Source: three-view drawing plus pictorial views. Frame: mm from the lowest corner of the part. Round coordinates to 2 decimals unless told otherwise and drop trailing zeros. Order: outer loops, then holes, each group sorted by start corner. A loop starts at its lowest first (then second) coordinate and runs counter-clockwise, first axis right, second up. Notation, with made-up numbers: (4, 61.25) - (58, 61.25) arc R15 ccw to (58, 70.25) - close; hole circle Ø9 at (20.5, 18.5). An arc over 180 degrees is marked (long way). Use one line per item in the form item = value. Start each with the question number.
Q1. Draft query along Z for the marked faces 1, 2 and 3. Return one class per face: released by +Z, released by -Z, zero draft, split by the parting line, or undercut.
Q2. Pin query (flat end, axial travel): pin 1 Ø1.5 at (y, z) = (8.5, 9) entering from -X; pin 2 Ø4 at (y, z) = (6, 8) entering from +X; pin 3 Ø1 at (y, z) = (4, 2.5) entering from -X; pin 4 Ø9.5 at (x, z) = (15.01, 13) entering from +Y. Return the tip coordinate at first contact, or that it passes through.
Q3. Cut plane A-A, the plane y = 5.5. Return the cut outline in (x, z) (1 decimal), and give its area (3 significant figures).
Q4. Cut plane B-B, the plane y = 11.5. Return the cut outline in (x, z) (1 decimal).
Q5. Ray query, line 1 (Z direction, x = 14, y = 3.5) (1 decimal); line 2 (Z direction, x = 11, y = 2.5); line 3 (X direction, y = 2.5, z = 13). Return the intervals inside material, ascending. Write a range as [from, to].
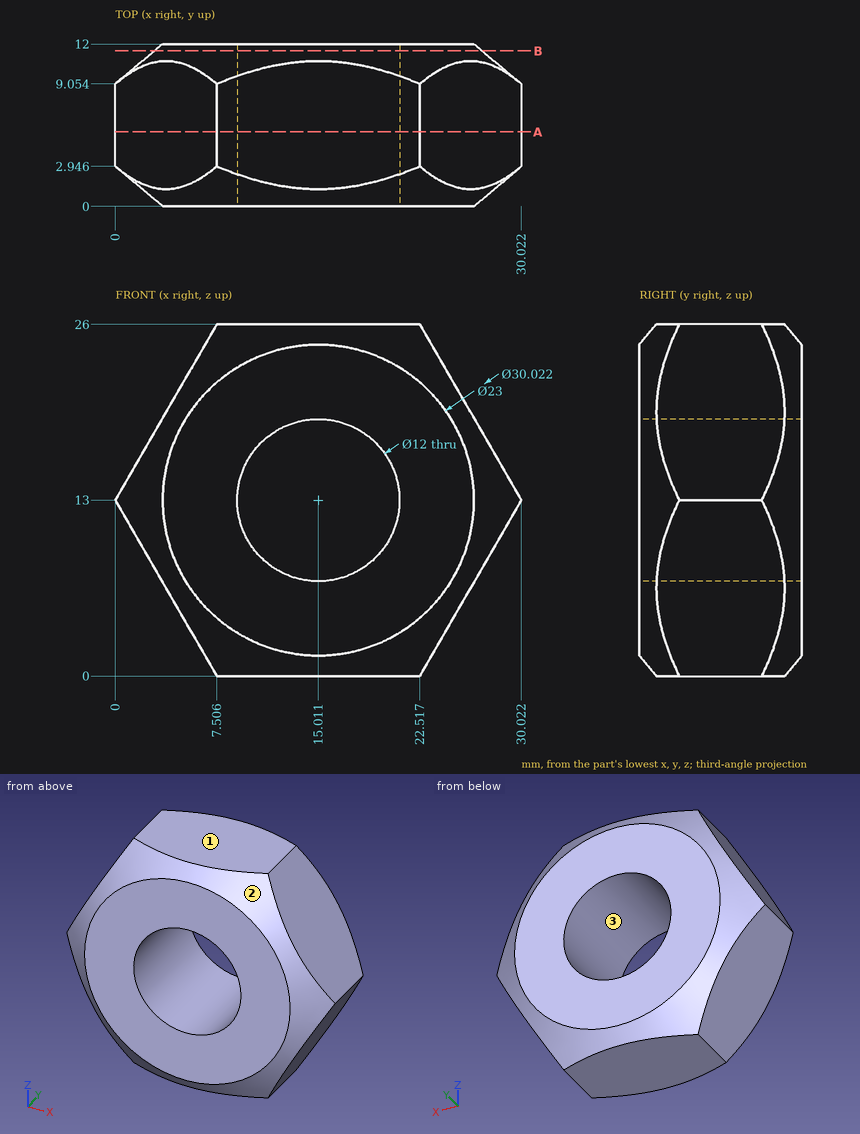
Completed:
q1.face_1 = released by +Z
q1.face_2 = split by the parting line
q1.face_3 = undercut
q2.pin_1 = 1.88
q2.pin_2 = 28.29
q2.pin_3 = 5.77
q2.pin_4 = through
q3.outline = (0, 13) - (7.5, 0) - (22.5, 0) - (30, 13) - (22.5, 26) - (7.5, 26) - close; hole circle Ø12 at (15, 13)
q3.area = 472 mm2
q4.outline = circle Ø24.2 at (15, 13); hole circle Ø12 at (15, 13)
q5.line_1 = [0, 7.1], [18.9, 26]
q5.line_2 = [0, 8.54], [17.46, 26]
q5.line_3 = [0.53, 9.01], [21.01, 29.49]
